Geometry check sheet. Reference: the model listing, model coordinates, mm. Round coordinates to 2 decimals unless told otherwise and drop trailing zeros. Write each loop counter-clockwise with the first axis right and the second up, starting at its lowest first coordinate (ties: lowest second). Pieces come first, ordered by that corner, then holes. Notation, with made-up numbers: (77.5, 44) - (85.5, 44) arc R20 cw to (85.5, 48) - close; hole circle Ø4 at (-5, 79.25). An arc over 180 degrees is marked (long way). Return JSON: item names as keys, results as strings. Group by question number.
from build123d import *

# Parameters (mm, degrees)
SKETCH1_R           = 40
BOSS_EXTRUDE1_DEPTH = 10


with BuildPart() as part:
    # Sketch1 → Boss-Extrude1 (new body)
    with BuildSketch(Plane.XY):
        with BuildLine():
            Line((149.303943499, 95), (50, 95))
            ThreePointArc((50, 95), (0, 45), (-50, 95))
            Line((-50, 95), (-149.303943499, 95))
            Line((-149.303943499, 95), (-158.434545849, 83.102548453))
            Line((-158.434545849, 83.102548453), (-136.818181818, -81.181818182))
            Line((-136.818181818, -81.181818182), (-123, -95))
            Line((-123, -95), (-50.051564514, -95))
            Line((-50.051564514, -95), (-50, -95))
            ThreePointArc((-50, -95), (0, -45), (50, -95))
            Line((50, -95), (123, -95))
            Line((123, -95), (136.818181818, -81.181818182))
            Line((136.818181818, -81.181818182), (158.434545849, 83.102548453))
            Line((158.434545849, 83.102548453), (149.303943499, 95))
        make_face()
        with Locations((-71.75, 0)):
            Circle(SKETCH1_R, mode=Mode.SUBTRACT)
        with Locations((71.75, 0)):
            Circle(SKETCH1_R, mode=Mode.SUBTRACT)
    extrude(amount=BOSS_EXTRUDE1_DEPTH)


solid = part.part
1. Section check A-A (x = -71.75). Enter the section's corners in (y, z), and give its area (3 significant figures).
2. Section check D-D (y = -68.5). Enter the section's corners in (x, z), and give its area (3 significant figures).
3. Depth check by flat-ended pin: pin 1 Ø2 at (y, z) = (59.5, 7) entering from +X. Enter the tip coordinate at first touch or a pass-through.
4. Mould release check, pull along Y, two halves, no side actions. Record for faces 1 (the face through (-33.597, 12.015, 4.93)), 2 (the face through (109.903, 12.015, 4.93)), 3 (the face through (100, 95, 5)), 4 (the face through (-130, -88, 5)): pulls with the +Y half, pulls with the -Y half, needs draft (parallel to the pull), parting line crosses it, or undercut.
5. Section check B-B (y = 16.5). Enter the section's corners in (x, z), and give its area (3 significant figures).
6. Material ranges on line 1 along Y through (x, z) = (-71.75, 7.25); line 2 along X through (y, z) = (-25.5, 1); line 3 along X through (y, z) = (73, 3.75), recorded low to high.
7. Section check C-C (z = 4). Enter the section's corners in (x, y).
Result sheet:
{
 "1": {"outline": "(-95, 0) - (-40, 0) - (-40, 10) - (-95, 10) - close; (40, 0) - (95, 0) - (95, 10) - (40, 10) - close", "area": "1,100 mm²"},
 "2": {"outline": "(-138.49, 0) - (-42.4, 0) - (-42.4, 10) - (-138.49, 10) - close; (42.4, 0) - (138.49, 0) - (138.49, 10) - (42.4, 10) - close", "area": "1,920 mm²"},
 "3": {"pin 1": "stops at x = 155.46"},
 "4": {"face 1": "undercut", "face 2": "undercut", "face 3": "pulls with the +Y half", "face 4": "pulls with the -Y half"},
 "5": {"outline": "(-149.67, 0) - (-108.19, 0) - (-108.19, 10) - (-149.67, 10) - close; (-35.31, 0) - (35.31, 0) - (35.31, 10) - (-35.31, 10) - close; (108.19, 0) - (149.67, 0) - (149.67, 10) - (108.19, 10) - close", "area": "1,540 mm²"},
 "6": {"line 1": "y = -95 to -40, 40 to 95", "line 2": "x = -144.14 to -102.57, -40.93 to 40.93, 102.57 to 144.14", "line 3": "x = -157.11 to -44.9, 44.9 to 157.11"},
 "7": {"outline": "(-158.43, 83.1) - (-136.82, -81.18) - (-123, -95) - (-50, -95) arc R50 cw to (50, -95) - (123, -95) - (136.82, -81.18) - (158.43, 83.1) - (149.3, 95) - (50, 95) arc R50 cw to (-50, 95) - (-149.3, 95) - close; hole circle Ø80 at (-71.75, 0); hole circle Ø80 at (71.75, 0)"}
}
